Model file for the job. Use its own axes, mm. A direction names the side the tool comes from. Round coordinates to 2 decimals unless told otherwise and drop trailing zeros. Order: outer loops, then holes, each group sorted by start corner. A loop starts at its lowest first (then second) coordinate and runs counter-clockwise, first axis right, second up. Notation, with made-up numbers: (16.5, 20) -> (28.5, 20) arc R18 ccw to (28.5, 34) -> close; hole circle Ø10 at (8.5, 9). An arc over 180 degrees is marked (long way). Put each result on its own line as item: value. Start each with the question number.
Q1. Flat gauge pins, fed straight in: P1, Ø1, axis at y = 0, z = -8.5, coming from the -X side; P2, Ø1.5, axis at x = -2.5, z = 7, coming from the -Y side. Where does each tip first touch, or does it go through?
Q2. Probe L1, parallel to Y at x = -0.15, z = -11; L2, parallel to Y at x = -0.9, z = 12. List the from-to ranges inside material, lowest first.
Q3. Cut at C-C, the plane z = 9.5. List the corners of the cut face in (x, y).
Q4. Cut at B-B, the plane z = -11. List the corners of the cut face in (x, y).
Q5. Cut at A-A, the plane y = 0. List the corners of the cut face in (x, z), and give its area (3 significant figures).
Q6. 3-axis set-ups, long thin cutter, end or side, ignore diameter. For faces 1 (the face through (-2.5, 0, -11)), 2 (the face through (0, 0, -16.5)): which of +Z, -Z, +X, -X, +Y, -Y reach the whole face in a straight line?
from build123d import *

# Parameters (mm, degrees)
SKETCH1_R           = 3
BOSS_EXTRUDE1_DEPTH = 16.5
CHAMFER1_SIZE       = 0.2
SKETCH2_W           = 0.5
SKETCH2_H           = 10
CUT_EXTRUDE1_DEPTH  = 15


with BuildPart() as part:
    # Sketch1 → Boss-Extrude1 (new, symmetric)
    with BuildSketch(Plane.XY):
        Circle(SKETCH1_R)
    extrude(amount=BOSS_EXTRUDE1_DEPTH, both=True)

    # Chamfer1
    chamfer1_edges = [part.edges().sort_by_distance(p)[0] for p in [
        (-3, 0, -16.5),
        (-3, 0, 16.5),
    ]]
    chamfer(chamfer1_edges, length=CHAMFER1_SIZE)

    # Sketch2 → Cut-Extrude1 (cut, symmetric)
    with BuildSketch(Plane(origin=(0, 0, 0), x_dir=(1, 0, 0), z_dir=(0, 1, 0))):
        with Locations((-2.75, 11.5)):
            Rectangle(SKETCH2_W, SKETCH2_H)
    extrude(amount=CUT_EXTRUDE1_DEPTH, both=True, mode=Mode.SUBTRACT)


solid = part.part
Ans:
1. P1: stops at x = -2.5
1. P2: stops at y = -2.44
2. L1: y = -3 to 3
2. L2: y = -2.86 to 2.86
3. outline: circle Ø6 at (0, 0)
4. outline: (-2.5, -1.66) arc R3 ccw (long way) to (-2.5, 1.66) -> close
5. outline: (-3, -6.5) -> (-2.5, -6.5) -> (-2.5, -16.5) -> (2.8, -16.5) -> (3, -16.3) -> (3, 16.3) -> (2.8, 16.5) -> (-2.8, 16.5) -> (-3, 16.3) -> close
5. area: 193 mm^2
6. face 1: -Z, -X, +Y, -Y
6. face 2: -Z, +X, -X, +Y, -Y
